Model file for the job. Use its own axes, mm. Face numbers are marked on the shaded views. A direction names the side the tool comes from. Coordinates: 2 decimals unless noted, no trailing zeros. Order: outer loops, then holes, each group sorted by start corner. A loop starts at its lowest first (then second) coordinate and runs counter-clockwise, first axis right, second up. Notation, with made-up numbers: M 74.25,-19 L 106.25,-19 A27 cw 106.25,-3 Z; hole C -3.5,75.5 d2. An arc over 180 degrees is marked long. Return JSON: item names as keys, results as strings.
```python
from build123d import *

# Parameters (mm, degrees)
SKETCH1_W           = 190
SKETCH1_H           = 95
BOSS_EXTRUDE1_DEPTH = 20
SHELL1_T            = -1
SKETCH2_W           = 146
SKETCH2_H           = 10
CUT_EXTRUDE1_DEPTH  = 1
SKETCH4_R           = 3.5
SKETCH4_W           = 9
SKETCH4_H           = 5.067595116
CUT_EXTRUDE2_DEPTH  = 10
SKETCH5_W           = 3
SKETCH5_H           = 2
CUT_EXTRUDE3_DEPTH  = 1
SKETCH6_R           = 2
CUT_EXTRUDE4_DEPTH  = 1
SKETCH8_W           = 3
SKETCH8_H           = 2
SKETCH8_W_2         = 27
SKETCH8_W_3         = 7
SKETCH8_W_4         = 17
SKETCH8_W_5         = 10
CUT_EXTRUDE5_DEPTH  = 1
SKETCH9_W           = 3
SKETCH9_H           = 2
SKETCH9_W_2         = 17
SKETCH9_W_3         = 6
SKETCH9_W_4         = 14
CUT_EXTRUDE6_DEPTH  = 1
SKETCH10_W          = 146
SKETCH10_H          = 12
BOSS_EXTRUDE2_DEPTH = 1
SKETCH11_R          = 3.5
SKETCH11_W          = 156
SKETCH11_H          = 11.148334169
SKETCH11_W_2        = 9
SKETCH11_H_2        = 5.067595116
BOSS_EXTRUDE3_DEPTH = 1
SKETCH12_W          = 22.5
SKETCH12_H          = 11
BOSS_EXTRUDE4_DEPTH = 1


with BuildPart() as part:
    # Sketch1 → Boss-Extrude1 (new body)
    with BuildSketch(Plane.XY):
        with Locations((67.138623448, 38.125260091)):
            Rectangle(SKETCH1_W, SKETCH1_H)
    extrude(amount=BOSS_EXTRUDE1_DEPTH)

    # Shell1
    shell1_openings = [part.faces().sort_by_distance(p)[0] for p in [
        (67.138623448, 38.125260091, 0),
    ]]
    offset(amount=SHELL1_T, openings=shell1_openings, kind=Kind.INTERSECTION)

    # Sketch2 → Cut-Extrude1 (cut)
    with BuildSketch(Plane(origin=(0, 85.625260091, 0), x_dir=(1, 0, 0), z_dir=(0, 1, 0))):
        Polygon((139.138623448, -9), (139.138623448, -8), (139.638623448, -8), (149.638623448, -8), (149.638623448, -19), (139.638623448, -19), (139.138623448, -19), (127.138623448, -19), (127.138623448, -9), align=None)
        with Locations((53.138623448, -14)):
            Rectangle(SKETCH2_W, SKETCH2_H)
    extrude(amount=-CUT_EXTRUDE1_DEPTH, mode=Mode.SUBTRACT)

    # Sketch4 → Cut-Extrude2 (cut)
    with BuildSketch(Plane.XZ.offset(9.374739909)):
        with Locations(Location((144.138623448, 6.5, 0), (0, 0, 270))):
            Circle(SKETCH4_R)
        Polygon((124.166122212, 9.851665831), (138.166122212, 9.851665831), (138.166122212, 19), (-17.833877788, 19), (-17.833877788, 9.851665831), (-14.833877788, 9.851665831), (-14.833877788, 7.851665831), (-11.833877788, 7.851665831), (-11.833877788, 9.851665831), (5.166122212, 9.851665831), (5.166122212, 7.851665831), (8.166122212, 7.851665831), (8.166122212, 9.851665831), (14.166122212, 9.851665831), (14.166122212, 7.851665831), (17.166122212, 7.851665831), (17.166122212, 9.851665831), (34.166122212, 9.851665831), (34.166122212, 7.851665831), (37.166122212, 7.851665831), (37.166122212, 9.851665831), (43.166122212, 9.851665831), (43.166122212, 7.851665831), (46.166122212, 7.851665831), (46.166122212, 9.851665831), (63.166122212, 9.851665831), (63.166122212, 7.851665831), (66.166122212, 7.851665831), (66.166122212, 9.851665831), (72.166122212, 9.851665831), (72.166122212, 7.851665831), (75.166122212, 7.851665831), (75.166122212, 9.851665831), (92.166122212, 9.851665831), (92.166122212, 7.851665831), (95.166122212, 7.851665831), (95.166122212, 9.851665831), (101.166122212, 9.851665831), (101.166122212, 7.851665831), (104.166122212, 7.851665831), (104.166122212, 9.851665831), (121.166122212, 9.851665831), (121.166122212, 7.851665831), (124.166122212, 7.851665831), align=None)
        with Locations((109.666122212, 4.317868273)):
            Rectangle(SKETCH4_W, SKETCH4_H)
    extrude(amount=-CUT_EXTRUDE2_DEPTH, mode=Mode.SUBTRACT)

    # Sketch5 → Cut-Extrude3 (cut)
    with BuildSketch(Plane(origin=(0, 85.625260091, 0), x_dir=(1, 0, 0), z_dir=(0, 1, 0))):
        with Locations((-15.361376552, -8)):
            Rectangle(SKETCH5_W, SKETCH5_H)
        with Locations((14.638623448, -8)):
            Rectangle(SKETCH5_W, SKETCH5_H)
        with Locations((24.638623448, -8)):
            Rectangle(SKETCH5_W, SKETCH5_H)
        with Locations((54.638623448, -8)):
            Rectangle(SKETCH5_W, SKETCH5_H)
        with Locations((64.638623448, -8)):
            Rectangle(SKETCH5_W, SKETCH5_H)
        with Locations((84.638623448, -8)):
            Rectangle(SKETCH5_W, SKETCH5_H)
        with Locations((94.638623448, -8)):
            Rectangle(SKETCH5_W, SKETCH5_H)
        with Locations((114.638623448, -8)):
            Rectangle(SKETCH5_W, SKETCH5_H)
    extrude(amount=-CUT_EXTRUDE3_DEPTH, mode=Mode.SUBTRACT)

    # Sketch6 → Cut-Extrude4 (cut)
    with BuildSketch(Plane.XY.offset(20)):
        with Locations((-21.861376552, -3.374739909)):
            Circle(SKETCH6_R)
        with Locations((-21.861376552, 79.625260091)):
            Circle(SKETCH6_R)
        with Locations((156.138623448, 79.625260091)):
            Circle(SKETCH6_R)
        with Locations((156.138623448, -3.374739909)):
            Circle(SKETCH6_R)
    extrude(amount=-CUT_EXTRUDE4_DEPTH, mode=Mode.SUBTRACT)

    # Sketch8 → Cut-Extrude5 (cut)
    with BuildSketch(Plane(origin=(0, 85.625260091, 0), x_dir=(1, 0, 0), z_dir=(0, 1, 0))):
        with Locations((-18.361376552, -8)):
            Rectangle(SKETCH8_W, SKETCH8_H)
        with Locations((-0.361376552, -8)):
            Rectangle(SKETCH8_W_2, SKETCH8_H)
        with Locations((19.638623448, -8)):
            Rectangle(SKETCH8_W_3, SKETCH8_H)
        with Locations((39.638623448, -8)):
            Rectangle(SKETCH8_W_2, SKETCH8_H)
        with Locations((59.638623448, -8)):
            Rectangle(SKETCH8_W_3, SKETCH8_H)
        with Locations((74.638623448, -8)):
            Rectangle(SKETCH8_W_4, SKETCH8_H)
        with Locations((89.638623448, -8)):
            Rectangle(SKETCH8_W_3, SKETCH8_H)
        with Locations((104.638623448, -8)):
            Rectangle(SKETCH8_W_4, SKETCH8_H)
        with Locations((121.138623448, -8)):
            Rectangle(SKETCH8_W_5, SKETCH8_H)
    extrude(amount=-CUT_EXTRUDE5_DEPTH, mode=Mode.SUBTRACT)

    # Sketch9 → Cut-Extrude6 (cut)
    with BuildSketch(Plane.XZ.offset(9.374739909)):
        with Locations((-16.333877788, 8.851665831)):
            Rectangle(SKETCH9_W, SKETCH9_H)
        with Locations((-3.333877788, 8.851665831)):
            Rectangle(SKETCH9_W_2, SKETCH9_H)
        with Locations((11.166122212, 8.851665831)):
            Rectangle(SKETCH9_W_3, SKETCH9_H)
        with Locations((25.666122212, 8.851665831)):
            Rectangle(SKETCH9_W_2, SKETCH9_H)
        with Locations((40.166122212, 8.851665831)):
            Rectangle(SKETCH9_W_3, SKETCH9_H)
        with Locations((54.666122212, 8.851665831)):
            Rectangle(SKETCH9_W_2, SKETCH9_H)
        with Locations((69.166122212, 8.851665831)):
            Rectangle(SKETCH9_W_3, SKETCH9_H)
        with Locations((83.666122212, 8.851665831)):
            Rectangle(SKETCH9_W_2, SKETCH9_H)
        with Locations((98.166122212, 8.851665831)):
            Rectangle(SKETCH9_W_3, SKETCH9_H)
        with Locations((112.666122212, 8.851665831)):
            Rectangle(SKETCH9_W_2, SKETCH9_H)
        with Locations((131.166122212, 8.851665831)):
            Rectangle(SKETCH9_W_4, SKETCH9_H)
    extrude(amount=-CUT_EXTRUDE6_DEPTH, mode=Mode.SUBTRACT)

    # Sketch10 → Boss-Extrude2 (add)
    with BuildSketch(Plane(origin=(0, 85.625260091, 0), x_dir=(1, 0, 0), z_dir=(0, 1, 0))):
        with Locations((53.138623448, -13)):
            Rectangle(SKETCH10_W, SKETCH10_H)
    extrude(amount=-BOSS_EXTRUDE2_DEPTH)

    # Sketch11 → Boss-Extrude3 (add)
    with BuildSketch(Plane.XZ.offset(9.374739909)):
        with Locations((144.138623448, 6.5)):
            Circle(SKETCH11_R)
        with Locations((60.166122212, 13.425832916)):
            Rectangle(SKETCH11_W, SKETCH11_H)
        with Locations((109.666122212, 4.317868273)):
            Rectangle(SKETCH11_W_2, SKETCH11_H_2)
    extrude(amount=-BOSS_EXTRUDE3_DEPTH)

    # Sketch12 → Boss-Extrude4 (add)
    with BuildSketch(Plane(origin=(0, 85.625260091, 0), x_dir=(1, 0, 0), z_dir=(0, 1, 0))):
        with Locations((138.388623448, -13.5)):
            Rectangle(SKETCH12_W, SKETCH12_H)
    extrude(amount=-BOSS_EXTRUDE4_DEPTH)


solid = part.part
```
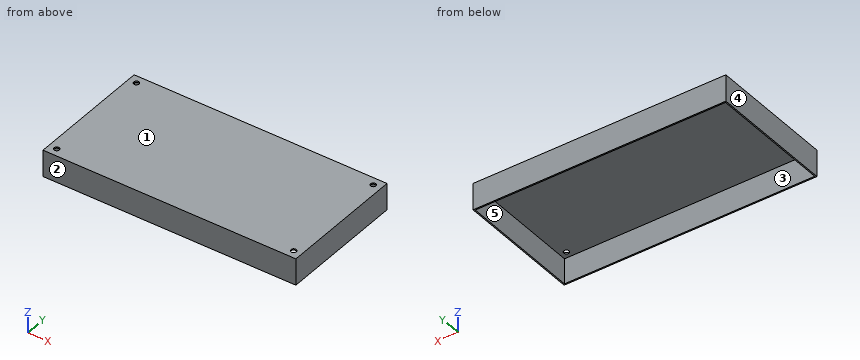
Item 1: Saw through at B-B (y = 28). Write the cut outline in (x, z), and give its area (3 significant figures).
Check result:
{"outline": "M -27.86,0 L -26.86,0 L -26.86,19 L 161.14,19 L 161.14,0 L 162.14,0 L 162.14,20 L -27.86,20 Z", "area": "228 mm2"}
Item 2: Wall check: line 1 (Y direction, x = 36, z = 15); line 2 (X direction, y = 61, z = 4); line 3 (Z direction, x = -1.5, y = 63.5). Give the ranges that are in metal, low to high.
Check result:
{"line 1": "y = -9.37 to -8.37, 84.63 to 85.63", "line 2": "x = -27.86 to -26.86, 161.14 to 162.14", "line 3": "z = 19 to 20"}
Item 3: 3-axis set-ups, long thin cutter, end or side, ignore diameter. For the marked faces 4 and 5: which of +Z, -Z, +X, -X, +Y, -Y reach the whole face in a straight line?
Check result:
{"face 4": "+Z, -Z, -X, +Y, -Y", "face 5": "-Z"}
Item 4: Saw through at C-C (x = 70.5). Write the cut outline in (y, z), and give its area (3 significant figures).
Check result:
{"outline": "M -9.37,0 L -8.37,0 L -8.37,19 L 84.63,19 L 84.63,0 L 85.63,0 L 85.63,20 L -9.37,20 Z", "area": "133 mm2"}
Item 5: Drop a flat-ended pin along its axis: pin 1 Ø5 at (x, y) = (156.14, 79.63) entering from -Z. Give the stop position or say it passes through.
Check result:
{"pin 1": "stops at z = 19"}
Item 6: Saw through at A-A (z = 5.25). Write the cut outline in (x, y).
Check result:
{"outline": "M -27.86,-9.37 L 162.14,-9.37 L 162.14,85.63 L -27.86,85.63 Z; hole M -26.86,-8.37 L 161.14,-8.37 L 161.14,84.63 L -26.86,84.63 Z"}
Item 7: Pull direction Y, two halves, no side cores. Call the marked faces 1, 2 and 3: +Y half, -Y half, draft (parallel to the pull), parting line (faces both ways), or undercut.
Check result:
{"face 1": "draft", "face 2": "-Y half", "face 3": "undercut"}
